The listing builds one solid part. Answer for the finished solid, in the listing's coordinates (mm). Give positions to 0.01 mm unless a question says otherwise; leave off trailing zeros. Write each loop counter-clockwise with the first axis right and the second up, starting at its lowest first coordinate (ties: lowest second). Pieces come first, ordered by that corner, then holes. Notation, with made-up numbers: (68.5, -21.5) - (78.5, -21.5) arc R21 ccw to (78.5, 11.5) - close; hole circle Ø6 at (65, 85.25). An arc over 180 degrees is marked (long way). One line per item, written item: value. Start each with the question number.
from build123d import *

# Parameters (mm, degrees)
SKETCH_1_W          = 360
SKETCH_1_H          = 50
SKETCH_1_R          = 2.5
EXTRUDE_1_DEPTH     = 20
HOLE_WIZARD_M10_1_D = 8.5


with BuildPart() as part:
    # 草图1 → 凸台-拉伸1 (new body)
    with BuildSketch(Plane.XZ.offset(-47)):
        with Locations((180, -25)):
            Rectangle(SKETCH_1_W, SKETCH_1_H)
        with Locations(Location((335, -25, 0), (0, 0, 90))):
            Circle(SKETCH_1_R, mode=Mode.SUBTRACT)
        with Locations(Location((65, -25, 0), (0, 0, 90))):
            Circle(SKETCH_1_R, mode=Mode.SUBTRACT)
        with Locations(Location((25, -25, 0), (0, 0, 90))):
            Circle(SKETCH_1_R, mode=Mode.SUBTRACT)
        with Locations(Location((295, -25, 0), (0, 0, 90))):
            Circle(SKETCH_1_R, mode=Mode.SUBTRACT)
    extrude(amount=-EXTRUDE_1_DEPTH)

    # M10 螺纹孔1 (through all)
    with Locations(Plane(origin=(0, 47, 0), x_dir=(-1, 0, 0), z_dir=(0, -1, 0))):
        with Locations((-335, 25), (-295, 25), (-65, 25), (-25, 25)):
            Hole(HOLE_WIZARD_M10_1_D / 2)


solid = part.part
Item 1: The mould has two halves that part along X. Classify faces 1 (the cylindrical face through (24.447, 57.14, -29.214)), 2 (the flat face through (360, 57, -25)), 3 (the flat face through (177, 67, -25)): +X half, -X half, draft (parallel to the pull), parting line (faces both ways), or undercut.
Item 2: Find section A-A on x = 335. Determine the outline of the cut face in (y, z).
Item 3: Straight lines are drawn through the part: line 1 along X through (y, z) = (64.5, -24.5); line 2 along Z through (x, y) = (335, 62.5); line 3 along X through (y, z) = (57.25, -21.5). For each, find the intervals that lie inside material, in ascending order.
Values:
1. face 1: undercut
1. face 2: +X half
1. face 3: draft
2. outline: (47, -50) - (67, -50) - (67, -29.25) - (47, -29.25) - close; (47, -20.75) - (67, -20.75) - (67, 0) - (47, 0) - close
3. line 1: 0 to 20.78, 29.22 to 60.78, 69.22 to 290.78, 299.22 to 330.78, 339.22 to 360
3. line 2: -50 to -29.25, -20.75 to 0
3. line 3: 0 to 22.59, 27.41 to 62.59, 67.41 to 292.59, 297.41 to 332.59, 337.41 to 360
